```python
from build123d import *

# Parameters (mm, degrees)
SKETCH_1_W          = 100
SKETCH_1_H          = 340
EXTRUDE_1_DEPTH     = 4
SKETCH_2_R          = 4.5
CUT_EXTRUDE_1_DEPTH = 14


with BuildPart() as part:
    # 草图1 → 凸台-拉伸1 (new, symmetric)
    with BuildSketch(Plane.XY):
        Rectangle(SKETCH_1_W, SKETCH_1_H)
    extrude(amount=EXTRUDE_1_DEPTH, both=True)

    # 草图2 → 切除-拉伸1 (cut, symmetric)
    with BuildSketch(Plane.XY):
        with Locations((-35, -125)):
            Circle(SKETCH_2_R)
        with Locations((35, 125)):
            Circle(SKETCH_2_R)
    extrude(amount=CUT_EXTRUDE_1_DEPTH, both=True, mode=Mode.SUBTRACT)


solid = part.part
```
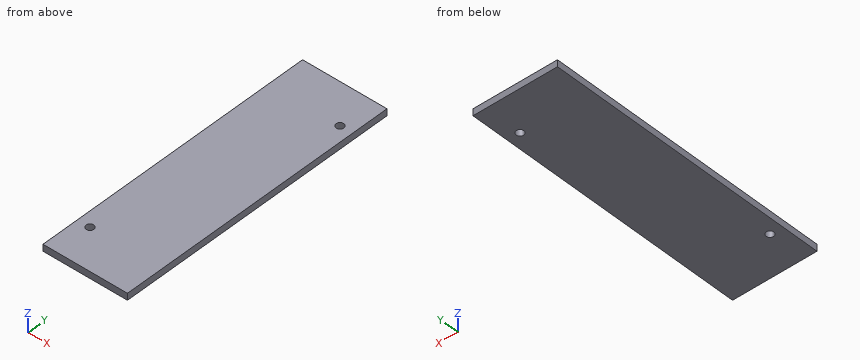
For this review, take the finished solid that the model builds, in its own axes (mm). Coordinates: 2 decimals unless noted, no trailing zeros. Write each loop counter-clockwise with the first axis right and the second up, starting at its lowest first coordinate (ties: lowest second). Pieces come first, ordered by that corner, then holes.
(1) Add section B-B on x = -35. Give the boundary of the cut face in (y, z), then the cut area to 3 significant figures.
(2) Wall thickness on probe 1 along Y at (x, z) = (35.5, 3.25); probe 2 along X at (y, z) = (-125, 1); probe 3 along Y at (x, z) = (-35, -2): over which ranges is each line inside the solid? List them lowest first.
(3) For pin 1 Ø8 at (x, y) = (-35, -125) entering from +Z, flat-tipped, find the tip position at first contact; note if it passes through.
(4) Add section A-A on y = -125. Give the boundary of the cut face in (x, z), then the cut area to 3 significant figures.
Answer sheet:
1. outline: (-170, -4) - (-129.5, -4) - (-129.5, 4) - (-170, 4) - close; (-120.5, -4) - (170, -4) - (170, 4) - (-120.5, 4) - close
1. area: 2,650 mm2
2. probe 1: y = -170 to 120.53, 129.47 to 170
2. probe 2: x = -50 to -39.5, -30.5 to 50
2. probe 3: y = -170 to -129.5, -120.5 to 170
3. pin 1: passes through
4. outline: (-50, -4) - (-39.5, -4) - (-39.5, 4) - (-50, 4) - close; (-30.5, -4) - (50, -4) - (50, 4) - (-30.5, 4) - close
4. area: 728 mm2
